```python
from build123d import *

# Parameters (mm, degrees)
SKETCH1_R             = 23.5
BOSS_EXTRUDE1_DEPTH   = 45
M6_TAPPED_HOLE1_D     = 5
M6_TAPPED_HOLE1_DEPTH = 15
M6_TAPPED_HOLE1_TIP   = 1.502151548
M5_TAPPED_HOLE1_D     = 4.2
M6_TAPPED_HOLE2_D     = 5
M6_TAPPED_HOLE2_DEPTH = 15
M6_TAPPED_HOLE2_TIP   = 1.502151548
M4_TAPPED_HOLE1_D     = 3.3
M4_TAPPED_HOLE1_DEPTH = 10.1
M4_TAPPED_HOLE1_TIP   = 0.991420021
CHAMFER1_SIZE         = 5
CHAMFER2_SIZE         = 2
SKETCH18_W            = 35
SKETCH18_H            = 15
CUT_EXTRUDE1_DEPTH    = 173.409396496
SKETCH19_W            = 20
SKETCH19_H            = 6
CUT_EXTRUDE2_DEPTH    = 2


with BuildPart() as part:
    # Sketch1 → Boss-Extrude1 (new body)
    with BuildSketch(Plane.XY):
        Polygon((-90, 140), (-90, -36), (-7.5, -36), (-7.5, -31), (7.5, -31), (7.5, -36), (40, -36), (40, 30), (-70, 30), (-70, 140), align=None)
        with Locations(Location((0, 0, 0), (0, 0, 180))):
            Circle(SKETCH1_R, mode=Mode.SUBTRACT)
    extrude(amount=BOSS_EXTRUDE1_DEPTH)

    # M6 Tapped Hole1
    with Locations(Plane.XZ.offset(36)):
        with Locations((-75, 10), (25, 10), (-75, 35), (25, 35)):
            Hole(M6_TAPPED_HOLE1_D / 2, depth=M6_TAPPED_HOLE1_DEPTH)
            with Locations((0, 0, -(M6_TAPPED_HOLE1_DEPTH + M6_TAPPED_HOLE1_TIP / 2))):  # 118° drill point
                Cone(0, M6_TAPPED_HOLE1_D / 2, M6_TAPPED_HOLE1_TIP, mode=Mode.SUBTRACT)

    # M5 Tapped Hole1 (through all)
    with Locations(Plane(origin=(-70, 0, 0), x_dir=(0, 0, -1), z_dir=(1, 0, 0))):
        with Locations((-22.5, 96), (-22.5, 36)):
            Hole(M5_TAPPED_HOLE1_D / 2)

    # M6 Tapped Hole2
    with Locations(Plane(origin=(0, 140, 0), x_dir=(-1, 0, 0), z_dir=(0, 1, 0))):
        with Locations((80, 7.5), (80, 37.5)):
            Hole(M6_TAPPED_HOLE2_D / 2, depth=M6_TAPPED_HOLE2_DEPTH)
            with Locations((0, 0, -(M6_TAPPED_HOLE2_DEPTH + M6_TAPPED_HOLE2_TIP / 2))):  # 118° drill point
                Cone(0, M6_TAPPED_HOLE2_D / 2, M6_TAPPED_HOLE2_TIP, mode=Mode.SUBTRACT)

    # M4 Tapped Hole1
    with Locations(Plane(origin=(0, 0, 0), x_dir=(-1, 0, 0), z_dir=(0, 0, -1))):
        with Locations((-19.445436483, 19.445436483), (19.445436483, -19.445436483), (-19.445436483, -19.445436483), (19.445436483, 19.445436483)):
            Hole(M4_TAPPED_HOLE1_D / 2, depth=M4_TAPPED_HOLE1_DEPTH)
            with Locations((0, 0, -(M4_TAPPED_HOLE1_DEPTH + M4_TAPPED_HOLE1_TIP / 2))):  # 118° drill point
                Cone(0, M4_TAPPED_HOLE1_D / 2, M4_TAPPED_HOLE1_TIP, mode=Mode.SUBTRACT)

    # Chamfer1
    chamfer1_edges = [part.edges().sort_by_distance(p)[0] for p in [
        (40, 30, 22.5),
    ]]
    chamfer(chamfer1_edges, length=CHAMFER1_SIZE)

    # Chamfer2
    chamfer2_edges = [part.edges().sort_by_distance(p)[0] for p in [
        (-80, 140, 45),
        (-80, 140, 0),
    ]]
    chamfer(chamfer2_edges, length=CHAMFER2_SIZE)

    # Sketch18 → Cut-Extrude1 (cut, through all)
    with BuildSketch(Plane(origin=(0, 0, 0), x_dir=(-1, 0, 0), z_dir=(0, 0, -1))):
        with Locations((52.5, 22.5)):
            Rectangle(SKETCH18_W, SKETCH18_H)
    extrude(amount=-CUT_EXTRUDE1_DEPTH, mode=Mode.SUBTRACT)

    # Sketch19 → Cut-Extrude2 (cut)
    with BuildSketch(Plane(origin=(0, 30, 0), x_dir=(1, 0, 0), z_dir=(0, 1, 0))):
        with Locations((0, -42)):
            Rectangle(SKETCH19_W, SKETCH19_H)
    extrude(amount=-CUT_EXTRUDE2_DEPTH, mode=Mode.SUBTRACT)


solid = part.part
```
Input: part model. Units: mm. Frame: model coordinates. A direction names the side the tool comes from. Give positions to 0.01 mm unless a question says otherwise; leave off trailing zeros. Order: outer loops, then holes, each group sorted by start corner. A loop starts at its lowest first (then second) coordinate and runs counter-clockwise, first axis right, second up.
1. Cut plane B-B (y = 74.5). Return loops of the section in (x, z).
Computed:
outline: (-90, 0) - (-70, 0) - (-70, 45) - (-90, 45) - close
2. Draft query along X for faces 4 (the face through (-90, 53, 22)), 5 (the face through (-72.5, -28.4, 35.1)), 6 (the face through (-49, -36, 22)), 7 (the face through (7.5, -33, 22)). Return one class per face: released by +X, released by -X, zero draft, split by the parting line, or undercut.
Computed:
face 4: released by -X
face 5: undercut
face 6: zero draft
face 7: undercut
3. Line query: probe 1 along X at (y, z) = (-28, 35); probe 2 along Z at (x, y) = (25, -26.75); probe 3 along Y at (x, z) = (-74.5, 22.5). Output: solid intervals per line, ascending.
Computed:
probe 1: x = -90 to -77.5, -72.5 to 22.5, 27.5 to 40
probe 2: z = 0 to 7.5, 12.5 to 32.5, 37.5 to 45
probe 3: y = -36 to 33.9, 38.1 to 93.9, 98.1 to 140
4. Set-up query: faces 1 (the face through (0, 30, 22)), 2 (the face through (26.84, -28.4, 36.69)), 3 (the face through (-7.5, -34, 22)). Return all of +Z, -Z, +X, -X, +Y, -Y with unobstructed straight access to the full face (end or side cutting, diameter ignored); none if empty.
Computed:
face 1: +Z, -Z, +X, +Y
face 2: -Y
face 3: +Z, -Z, -Y
5. Cut plane A-A (x = 0). Return loops of the section in (y, z), and give its area (3 significant figures).
Computed:
outline: (-31, 0) - (-23.5, 0) - (-23.5, 45) - (-31, 45) - close; (23.5, 0) - (30, 0) - (30, 39) - (28, 39) - (28, 45) - (23.5, 45) - close
area: 618 mm2
6. Pin query (flat end, axial travel): pin 1 Ø7.5 at (x, z) = (-2.5, 20.5) entering from -Y; pin 2 Ø2 at (y, z) = (29, 41.5) entering from +X; pin 3 Ø2 at (x, y) = (19.45, -19.45) entering from -Z. Return the tip coordinate at first contact, or that it passes through.
Computed:
pin 1: stops at y = -31
pin 2: stops at x = 37
pin 3: stops at z = 10.49
7. Cut plane C-C (x = -52.5). Return loops of the section in (y, z).
Computed:
outline: (-36, 0) - (15, 0) - (15, 45) - (-36, 45) - close
